Source: CAD feature listing. Evaluate the final solid. Frame: model axes, mm. Face numbers are marked on the shaded views. A direction names the side the tool comes from. Give positions to 0.01 mm unless a question says otherwise; leave off trailing zeros. Order: outer loops, then holes, each group sorted by start corner. A loop starts at its lowest first (then second) coordinate and runs counter-clockwise, first axis right, second up.
```python
from build123d import *

# Parameters (mm, degrees)
SKETCH1_R           = 6.35
BOSS_EXTRUDE1_DEPTH = 25.4
SKETCH2_R           = 22.23
CUT_EXTRUDE1_DEPTH  = 12.7
CUT_EXTRUDE_1_REACH = 169.736
SCALE_1_SCALE       = 0.5
SCALE_2_SCALE       = 0.5
SKETCH_2_R          = 0.75
CUT_EXTRUDE_2_DEPTH = 18.517255065
SKETCH_3_W          = 3.175
SKETCH_3_H          = 0.9525
CUT_EXTRUDE_3_DEPTH = 6.35
CUT_EXTRUDE_4_DEPTH = 1.5
CUT_EXTRUDE_5_DEPTH = 1.5


with BuildPart() as part:
    # Sketch1 → Boss-Extrude1 (new body)
    with BuildSketch(Plane.XY):
        with BuildLine():
            Line((0, -15.24), (165.1, -15.24))
            Line((165.1, -15.24), (165.1, -6.98))
            Line((165.1, -6.98), (27.790517271, -2.185047205))
            Line((27.790517271, -2.185047205), (22.140950977, -1.987760002))
            Line((22.140950977, -1.987760002), (15.139966118, -1.743280224))
            ThreePointArc((15.139966118, -1.743280224), (11.375965687, 10.14125262), (0, 15.24))
            Line((0, 15.24), (-24, 15.24))
            Line((-24, 15.24), (-63.5, 8.26))
            Line((-63.5, 8.26), (-63.5, 0))
            Line((-63.5, 0), (-50.8, 0))
            Line((-50.8, 0), (-50.8, 3.81))
            Line((-50.8, 3.81), (-46.99, 3.81))
            Line((-46.99, 3.81), (-21.901068467, 3.81))
            ThreePointArc((-21.901068467, 3.81), (-17.369676473, 1.405708043), (-14.920995783, -3.10185184))
            ThreePointArc((-14.920995783, -3.10185184), (-9.617311942, -11.82222107), (0, -15.24))
        make_face()
        Circle(SKETCH1_R, mode=Mode.SUBTRACT)
    extrude(amount=BOSS_EXTRUDE1_DEPTH)

    # Sketch2 → Cut-Extrude1 (cut)
    with BuildSketch(Plane.XY.offset(25.4)):
        Circle(SKETCH2_R)
    extrude(amount=-CUT_EXTRUDE1_DEPTH, mode=Mode.SUBTRACT)

    # 草图1 → 切除-拉伸1 (cut, up to next)
    with BuildSketch(Plane.XY.offset(25.4), mode=Mode.PRIVATE) as cut_extrude_1_sk1:
        Polygon((43.109053356, -15.24), (43.109053356, -2.719982272), (165.1, -6.98), (165.1, -15.24), align=None)
    cut_extrude_1_tool1 = extrude(cut_extrude_1_sk1.sketch, amount=-CUT_EXTRUDE_1_REACH, mode=Mode.PRIVATE) & part.part
    add(cut_extrude_1_tool1.solids().sort_by_distance((99.936391, -9.972218, 25.4))[0], mode=Mode.SUBTRACT)


with BuildPart() as part_1:
    # 缩放比例1: scaled about (0, 0, 0)
    add(part.part.scale(SCALE_1_SCALE))


with BuildPart() as part_2:
    # 缩放比例2: scaled about (0, 0, 0)
    add(part_1.part.scale(SCALE_2_SCALE))

    # 草图2 → 切除-拉伸2 (cut, through all)
    with BuildSketch(Plane.XY.offset(6.35)):
        with Locations((8.277263339, -2.244997784)):
            Circle(SKETCH_2_R)
    extrude(amount=-CUT_EXTRUDE_2_DEPTH, mode=Mode.SUBTRACT)

    # 草图3 → 切除-拉伸3 (cut)
    with BuildSketch(Plane.XY.offset(6.35)):
        with Locations((-14.2875, 0.47625)):
            Rectangle(SKETCH_3_W, SKETCH_3_H)
    extrude(amount=-CUT_EXTRUDE_3_DEPTH, mode=Mode.SUBTRACT)

    # 草图4 → 切除-拉伸4 (cut)
    with BuildSketch(Plane.XY.offset(6.35)):
        Polygon((-15.875, 2.065), (-15.875, 0.9525), (-12.675, 0.9525), (-12.675, 2.630468354), align=None)
    extrude(amount=-CUT_EXTRUDE_4_DEPTH, mode=Mode.SUBTRACT)

    # 草图5 → 切除-拉伸5 (cut)
    with BuildSketch(Plane(origin=(0, 0, 0), x_dir=(-1, 0, 0), z_dir=(0, 0, -1))):
        Polygon((15.875, 2.065), (15.875, 0.9525), (12.675, 0.9525), (12.675, 2.630468354), align=None)
    extrude(amount=-CUT_EXTRUDE_5_DEPTH, mode=Mode.SUBTRACT)


solid = part_2.part
```
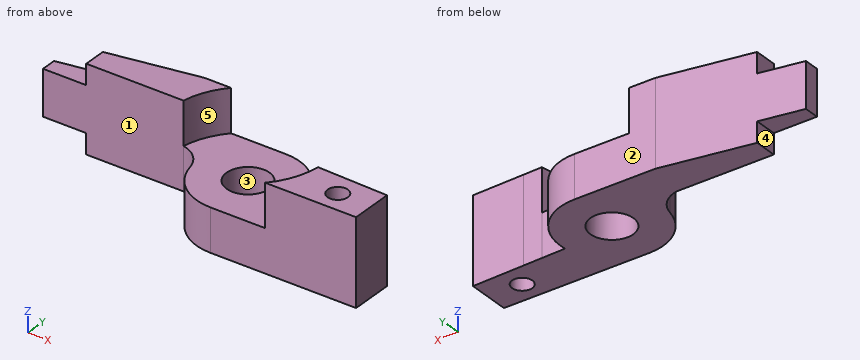
1) Section query C-C, the plane y = -2.75. Return the cut outline in (x, z) (3 decimals).
Report:
outline: (-2.637, 0) - (7.723, 0) - (7.723, 6.35) - (4.829, 6.35) - (4.829, 3.175) - (-2.637, 3.175) - close; (8.832, 0) - (10.777, 0) - (10.777, 6.35) - (8.832, 6.35) - close
2) Material intervals for L1, parallel to Z at x = -0.5, y = 2.5 (3 decimals); L2, parallel to X at y = -1.25, z = 3; L3, parallel to X at y = -2.5, z = 6.25, sorted ascending.
Report:
L1: z = 0 to 3.175
L2: x = -3.6 to -0.98, 0.98 to 10.78
L3: x = 4.96 to 7.57, 8.98 to 10.78
3) Section query D-D, the plane x = -6.5. Return the cut outline in (y, z).
Report:
outline: (0.95, 0) - (3.72, 0) - (3.72, 6.35) - (0.95, 6.35) - close
4) Reachability of the marked faces 1, 2, 3, 4 and 5 from +Z, -Z, +X, -X, +Y, -Y: full face, straight path, thin tool, end or side. Return the list, or none.
Report:
face 1: +Z, -Z, -X, -Y
face 2: +Z, -Z, +X, -X, +Y
face 3: +Z, -Z
face 4: -Z, -X, +Y, -Y
face 5: +Z, +X, -Y
5) Section query A-A, the plane z = 3.5. Count the separate pieces of the cut face and the enclosed holes in it, and give its area (3 significant figures).
Report:
separate pieces: 2
enclosed holes: 1
area: 39.5 mm2
6) Pin query (flat end, axial travel): pin 1 (3 mm diameter, centred on x = -10, z = 4, fed in from -Y); pin 2 (2.5 mm diameter, centred on x = 1, y = -0.5, fed in from +Z) (3 decimals); pin 3 (0.5 mm diameter, centred on x = -14.5, y = 2, fed in from -Z). Return the tip coordinate at first contact, or that it passes through.
Report:
pin 1: stops at y = 0.95
pin 2: stops at z = 3.175
pin 3: stops at z = 1.5
7) Section query B-B, the plane y = 0. Return the cut outline in (x, z) (1 decimal), and give its area (3 significant figures).
Report:
outline: (-4.1, 0) - (-1.6, 0) - (-1.6, 3.2) - (-4.1, 3.2) - close; (1.6, 0) - (3.8, 0) - (3.8, 3.2) - (1.6, 3.2) - close
area: 14.9 mm2
